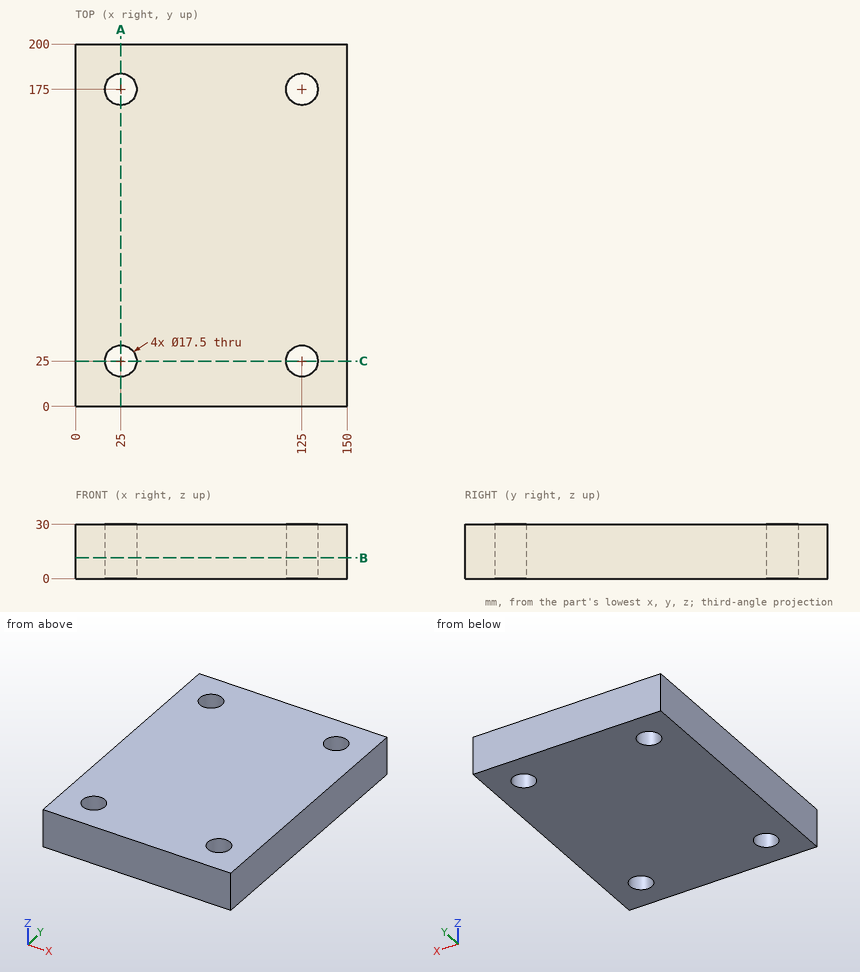
Drawing for the job (mm, zero at the part's lowest x, y, z). Give positions to 0.01 mm unless a question says otherwise; leave off trailing zeros. Order: outer loops, then holes, each group sorted by start corner. A loop starts at its lowest first (then second) coordinate and runs counter-clockwise, first axis right, second up. Notation, with made-up numbers: (0, -5.75) - (41, -5.75) arc R25 ccw to (41, 13.25) - close; hole circle Ø9 at (14.5, 43). An arc over 180 degrees is marked (long way). Use one line per item in the form item = value.
Item 1: Slice it at A-A on x = 25. Give the cut face in (y, z).
Solution:
outline = (0, 0) - (16.25, 0) - (16.25, 30) - (0, 30) - close; (33.75, 0) - (166.25, 0) - (166.25, 30) - (33.75, 30) - close; (183.75, 0) - (200, 0) - (200, 30) - (183.75, 30) - close
Item 2: Slice it at B-B on z = 11.5. Give the cut face in (x, y), and give its area (3 significant figures).
Solution:
outline = (0, 0) - (150, 0) - (150, 200) - (0, 200) - close; hole circle Ø17.5 at (25, 25); hole circle Ø17.5 at (25, 175); hole circle Ø17.5 at (125, 25); hole circle Ø17.5 at (125, 175)
area = 29,000 mm2
Item 3: Slice it at C-C on y = 25. Give the cut face in (x, z), and give its area (3 significant figures).
Solution:
outline = (0, 0) - (16.25, 0) - (16.25, 30) - (0, 30) - close; (33.75, 0) - (116.25, 0) - (116.25, 30) - (33.75, 30) - close; (133.75, 0) - (150, 0) - (150, 30) - (133.75, 30) - close
area = 3,450 mm2
Item 4: Probe probe 1 along Y at (x, z) = (25, 21.75); probe 2 along Y at (x, z) = (29, 16.25); probe 3 along X at (y, z) = (178, 13.25). List the from-to ranges inside material, lowest first. Write a range as from..to.
Solution:
probe_1 = 0..16.25, 33.75..166.25, 183.75..200
probe_2 = 0..17.22, 32.78..167.22, 182.78..200
probe_3 = 0..16.78, 33.22..116.78, 133.22..150
